The listing builds one solid part. Answer for the finished solid, in the listing's coordinates (mm). Coordinates: 2 decimals unless noted, no trailing zeros. Order: outer loops, then holes, each group sorted by start corner. A loop starts at its lowest first (then second) coordinate and runs counter-clockwise, first axis right, second up. Notation, with made-up numbers: (18, -29.5) -> (70, -29.5) arc R19 cw to (70, 2.5) -> close; hole circle Ø3 at (60, 40.5). An arc over 180 degrees is marked (long way). Write item = value, one per line. Start each with the question number.
```python
from build123d import *

# Parameters (mm, degrees)
BOSS_EXTRUDE1_DEPTH = 10


with BuildPart() as part:
    # Sketch1 → Boss-Extrude1 (new body)
    with BuildSketch(Plane(origin=(0, 0, 0), x_dir=(0, 0, -1), z_dir=(1, 0, 0))):
        with BuildLine():
            Line((0, -158), (0, 158))
            Line((0, 158), (35, 170))
            Line((35, 170), (535.799605091, 170))
            ThreePointArc((535.799605091, 170), (536.59744846, 169.968121486), (537.390205017, 169.872689192))
            Line((537.390205017, 169.872689192), (985.809794983, 97.627310808))
            ThreePointArc((985.809794983, 97.627310808), (986.60255154, 97.531878514), (987.400394909, 97.5))
            Line((987.400394909, 97.5), (1403, 97.5))
            Line((1403, 97.5), (1438, 85.5))
            Line((1438, 85.5), (1438, -85.5))
            Line((1438, -85.5), (1403, -97.5))
            Line((1403, -97.5), (987.400394909, -97.5))
            ThreePointArc((987.400394909, -97.5), (986.60255154, -97.531878514), (985.809794983, -97.627310808))
            Line((985.809794983, -97.627310808), (537.390205017, -169.872689192))
            ThreePointArc((537.390205017, -169.872689192), (536.59744846, -169.968121486), (535.799605091, -170))
            Line((535.799605091, -170), (35, -170))
            Line((35, -170), (0, -158))
        make_face()
    extrude(amount=BOSS_EXTRUDE1_DEPTH)


solid = part.part
```
Item 1: Each of these flat-tipped pins is pushed along its axis until it touches: pin 1 (3 mm diameter, centred on x = 4, z = -1114.5, fed in from +Y); pin 2 (6 mm diameter, centred on x = 7.5, z = -557.5, fed in from +Y). Where does it stop, or does it pass through?
Item 2: Section B-B, the plane z = -596 is taken. Give the vertices of the cut face in (x, y).
Item 3: Consider probe 1 along Y at (x, z) = (8, -616.5); probe 2 along Y at (x, z) = (6, -983.5). Determine where each line is inside the solid, lowest interval first.
Item 4: Section A-A, the plane x = 6.25 is taken. Give the vertices of the cut face in (y, z), then the cut area to 3 significant figures.
Item 5: Section C-C, the plane y = 139 is taken. Give the vertices of the cut face in (x, z), then the cut area to 3 significant figures.
A:
q1.pin_1 = 97.5
q1.pin_2 = 167.12
q2.outline = (0, -160.43) -> (10, -160.43) -> (10, 160.43) -> (0, 160.43) -> close
q3.probe_1 = -157.13 to 157.13
q3.probe_2 = -98 to 98
q4.outline = (-170, -535.8) arc R10 ccw to (-169.87, -537.39) -> (-97.63, -985.81) arc R10 cw to (-97.5, -987.4) -> (-97.5, -1403) -> (-85.5, -1438) -> (85.5, -1438) -> (97.5, -1403) -> (97.5, -987.4) arc R10 cw to (97.63, -985.81) -> (169.87, -537.39) arc R10 ccw to (170, -535.8) -> (170, -35) -> (158, 0) -> (-158, 0) -> (-170, -35) -> close
q4.area = 390,000 mm^2
q5.outline = (0, -729.01) -> (10, -729.01) -> (10, 0) -> (0, 0) -> close
q5.area = 7,290 mm^2
